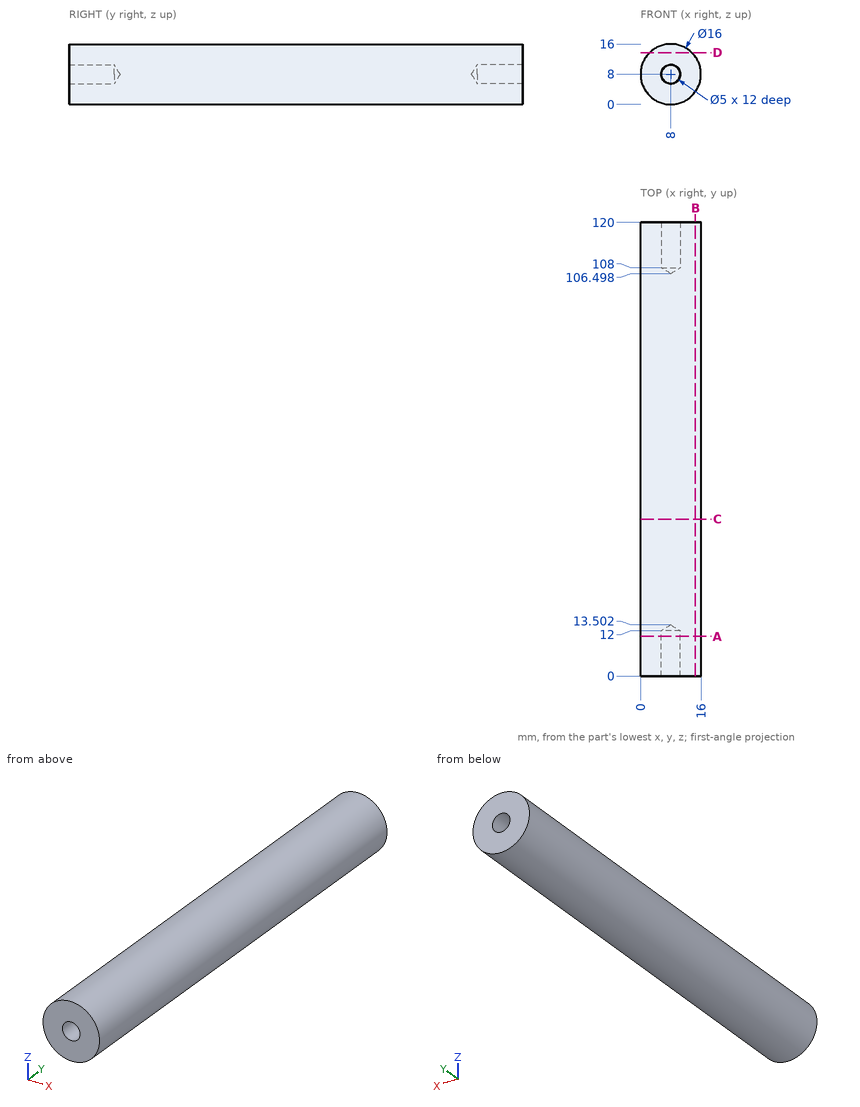
For this review, use the dimensioned drawing (mm, ordinates from the lowest corner) and the shaded views. Coordinates: 2 decimals unless noted, no trailing zeros. Order: outer loops, then holes, each group sorted by start corner. A loop starts at its lowest first (then second) coordinate and runs counter-clockwise, first axis right, second up. Notation, with made-up numbers: (-1, 67) - (5, 67) arc R26 ccw to (5, 81) - close; hole circle Ø2 at (73.25, 17). An arc over 180 degrees is marked (long way). Answer as a JSON object with one key per item and string values. Group by question number.
1. For probe 1 along Z at (x, y) = (8, 117); probe 2 along Z at (x, y) = (8.5, 84); probe 3 along Z at (x, y) = (2.25, 56.5), list the stretches that pass through material, from the lowest coordinate up.
2. We need section A-A on y = 10.5. State the section outline as (x, z) points.
3. We need section B-B on x = 14.5. State the section outline as (y, z) points.
4. We need section C-C on y = 41.5. State the section outline as (x, z) points, then the cut area to 3 significant figures.
5. Clearance check with flat-ended pins moving along their axes: P1, Ø4, axis at x = 8, z = 8, coming from the +Y side; P2, Ø8, axis at y = 19, z = 7, coming from the -X side; P3, Ø3, axis at x = 8, z = 8, coming from the +Y side; P4, Ø3, axis at y = 22, z = 10.5, coming from the -X side. State where each tip first meets the part, or that it passes through.
6. We need section D-D on z = 13.75. State the section outline as (x, y) points.
Final values:
{
 "1": {"probe 1": "0 to 5.5, 10.5 to 16", "probe 2": "0.02 to 15.98", "probe 3": "2.44 to 13.56"},
 "2": {"outline": "circle Ø16 at (8, 8); hole circle Ø5 at (8, 8)"},
 "3": {"outline": "(0, 3.34) - (120, 3.34) - (120, 12.66) - (0, 12.66) - close"},
 "4": {"outline": "circle Ø16 at (8, 8)", "area": "201 mm²"},
 "5": {"P1": "y = 107.7", "P2": "x = 0", "P3": "y = 107.4", "P4": "x = 0.06"},
 "6": {"outline": "(2.44, 0) - (13.56, 0) - (13.56, 120) - (2.44, 120) - close"}
}
